from build123d import *

# Parameters (mm, degrees)
BOSS_EXTRUDE1_DEPTH = 6
SKETCH2_R           = 2.5
BOSS_EXTRUDE2_DEPTH = 33
SKETCH3_R           = 6
BOSS_EXTRUDE3_DEPTH = 1
SKETCH4_R           = 3.704648002
CUT_EXTRUDE1_DEPTH  = 0.2


with BuildPart() as part:
    # Sketch1 → Boss-Extrude1 (new body)
    with BuildSketch(Plane.XY):
        with BuildLine():
            ThreePointArc((-8.5, -2.958039892), (-8.314915793, -3.444150891), (-8.102057706, -3.918757574))
            ThreePointArc((-8.102057706, -3.918757574), (-8.485281374, -8.485281374), (-3.918757574, -8.102057706))
            ThreePointArc((-3.918757574, -8.102057706), (-3.444150891, -8.314915793), (-2.958039892, -8.5))
            ThreePointArc((-2.958039892, -8.5), (0, -12), (2.958039892, -8.5))
            ThreePointArc((2.958039892, -8.5), (3.444150891, -8.314915793), (3.918757574, -8.102057706))
            ThreePointArc((3.918757574, -8.102057706), (8.485281374, -8.485281374), (8.102057706, -3.918757574))
            ThreePointArc((8.102057706, -3.918757574), (8.314915793, -3.444150891), (8.5, -2.958039892))
            ThreePointArc((8.5, -2.958039892), (12, 0), (8.5, 2.958039892))
            ThreePointArc((8.5, 2.958039892), (8.314915793, 3.444150891), (8.102057706, 3.918757574))
            ThreePointArc((8.102057706, 3.918757574), (8.485281374, 8.485281374), (3.918757574, 8.102057706))
            ThreePointArc((3.918757574, 8.102057706), (3.444150891, 8.314915793), (2.958039892, 8.5))
            ThreePointArc((2.958039892, 8.5), (0, 12), (-2.958039892, 8.5))
            ThreePointArc((-2.958039892, 8.5), (-3.444150891, 8.314915793), (-3.918757574, 8.102057706))
            ThreePointArc((-3.918757574, 8.102057706), (-8.485281374, 8.485281374), (-8.102057706, 3.918757574))
            ThreePointArc((-8.102057706, 3.918757574), (-8.314915793, 3.444150891), (-8.5, 2.958039892))
            ThreePointArc((-8.5, 2.958039892), (-12, 0), (-8.5, -2.958039892))
        make_face()
    extrude(amount=BOSS_EXTRUDE1_DEPTH)

    # Sketch2 → Boss-Extrude2 (add)
    with BuildSketch(Plane.XY.offset(6)):
        Circle(SKETCH2_R)
    extrude(amount=BOSS_EXTRUDE2_DEPTH)

    # Sketch3 → Boss-Extrude3 (add, symmetric)
    with BuildSketch(Plane.XY.offset(6)):
        Circle(SKETCH3_R)
    extrude(amount=BOSS_EXTRUDE3_DEPTH, both=True)

    # Sketch4 → Cut-Extrude1 (cut)
    with BuildSketch(Plane(origin=(0, 0, 0), x_dir=(-1, 0, 0), z_dir=(0, 0, -1))):
        Circle(SKETCH4_R)
    extrude(amount=-CUT_EXTRUDE1_DEPTH, mode=Mode.SUBTRACT)


solid = part.part
The listing builds one solid part. Answer for the finished solid, in the listing's coordinates (mm). A direction names the side the tool comes from. Coordinates: 2 decimals unless noted, no trailing zeros. Write each loop counter-clockwise with the first axis right and the second up, starting at its lowest first coordinate (ties: lowest second). Pieces come first, ordered by that corner, then holes. Notation, with made-up numbers: (69.5, 35) - (77.5, 35) arc R16 cw to (77.5, 55) - close; hole circle Ø7 at (1.25, 25). An arc over 180 degrees is marked (long way). Return JSON: item names as keys, results as strings.
1. The part is cut by section C-C on z = 22.5. Determine the outline of the cut face in (x, y).
Final values:
{"outline": "circle Ø5 at (0, 0)"}
2. The part is cut by section B-B on x = 4.75. Determine the outline of the cut face in (y, z), then the cut area to 3 significant figures.
Final values:
{"outline": "(-8.89, 0) - (8.89, 0) - (8.89, 6) - (3.67, 6) - (3.67, 7) - (-3.67, 7) - (-3.67, 6) - (-8.89, 6) - close", "area": "114 mm^2"}
3. The part is cut by section A-A on y = 0. Determine the outline of the cut face in (x, z), then the cut area to 3 significant figures.
Final values:
{"outline": "(-12, 0) - (-3.7, 0) - (-3.7, 0.2) - (3.7, 0.2) - (3.7, 0) - (12, 0) - (12, 6) - (6, 6) - (6, 7) - (2.5, 7) - (2.5, 39) - (-2.5, 39) - (-2.5, 7) - (-6, 7) - (-6, 6) - (-12, 6) - close", "area": "315 mm^2"}
4. Consider line 1 along Z through (x, y) = (9.25, -0.75); line 2 along Z through (x, y) = (-0.5, -2.5); line 3 along Y through (x, z) = (-4.25, 4.5). Determine where each line is inside the solid, lowest interval first.
Final values:
{"line 1": "0 to 6", "line 2": "0.2 to 7", "line 3": "-8.49 to 8.49"}
5. Which of the six approach directions +Z, -Z, +X, -X, +Y, -Y give full straight-line access (tool end or side, diameter ignored) to faces 4 (the face through (-6, -2, 6)), 5 (the face through (0, 0, 0.2)), 6 (the face through (8.43, -8.54, 2.96))?
Final values:
{"face 4": "+Z", "face 5": "-Z", "face 6": "+Z, -Z"}
6. Each of these flat-tipped pins is pushed along its axis until it touches: pin 1 Ø1.5 at (y, z) = (2.5, 25.5) entering from +X; pin 2 Ø1 at (y, z) = (2, 28) entering from +X; pin 3 Ø1 at (x, y) = (-6.5, -2) entering from -Z; pin 4 Ø6 at (x, y) = (-5.5, 1) entering from +Z. Where does it stop, or does it pass through?
Final values:
{"pin 1": "x = 1.79", "pin 2": "x = 2", "pin 3": "z = 0", "pin 4": "z = 7"}
7. For a pull along Y with two mould halves and no side action, classify faces 1 (the face through (-8.318, -3.437, 2.958)), 2 (the face through (-5.994, 0.264, 6.507)), 3 (the face through (0, 0, 39)) as +Y half, -Y half, draft (parallel to the pull), parting line (faces both ways), or undercut.
Final values:
{"face 1": "undercut", "face 2": "parting line", "face 3": "draft"}
